from build123d import *

# Parameters (mm, degrees)
EXTRUDE_1_DEPTH     = 20
FILLET_1_R          = 2
SKETCH_2_R          = 1.5
CUT_EXTRUDE_1_DEPTH = 60.760642304
SKETCH_3_R          = 1.5
CUT_EXTRUDE_2_DEPTH = 60.760642304


with BuildPart() as part:
    # 草图1 → 凸台-拉伸1 (new body)
    with BuildSketch(Plane(origin=(0, 0, 0), x_dir=(1, 0, 0), z_dir=(0, 1, 0))):
        Polygon((0, 45), (0, 0), (40.249223595, 0), align=None)
    extrude(amount=EXTRUDE_1_DEPTH)

    # 圆角1
    fillet_1_edges = [part.edges().sort_by_distance(p)[0] for p in [
        (40.249223595, 10, 0),
        (0, 10, 0),
        (0, 10, -45),
    ]]
    fillet(fillet_1_edges, radius=FILLET_1_R)

    # 草图2 → 切除-拉伸1 (cut, through all)
    with BuildSketch(Plane.ZY):
        with Locations((-20, 15)):
            Circle(SKETCH_2_R)
        with Locations((-20, 5)):
            Circle(SKETCH_2_R)
    extrude(amount=-CUT_EXTRUDE_1_DEPTH, mode=Mode.SUBTRACT)

    # 草图3 → 切除-拉伸2 (cut, through all)
    with BuildSketch(Plane.XY):
        with Locations((15, 15)):
            Circle(SKETCH_3_R)
        with Locations((15, 5)):
            Circle(SKETCH_3_R)
    extrude(amount=-CUT_EXTRUDE_2_DEPTH, mode=Mode.SUBTRACT)


solid = part.part
Verification items for the finished model (mm, model axes). Round coordinates to 2 decimals unless told otherwise and drop trailing zeros. Write each loop counter-clockwise with the first axis right and the second up, starting at its lowest first coordinate (ties: lowest second). Pieces come first, ordered by that corner, then holes.
(1) Section check D-D (y = 15). Enter the section's corners in (x, z), plus the area to 3 significant figures.
Returned:
outline: (0, -39.76) arc R2 ccw to (3.49, -41.1) - (13.5, -29.91) - (13.5, -21.5) - (0, -21.5) - close; (0, -18.5) - (13.5, -18.5) - (13.5, 0) - (2, 0) arc R2 ccw to (0, -2) - close; (16.5, -26.55) - (21.02, -21.5) - (16.5, -21.5) - close; (16.5, -18.5) - (23.7, -18.5) - (37.27, -3.33) arc R2 ccw to (35.78, 0) - (16.5, 0) - close
area: 752 mm2
(2) Mould release check, pull along X, two halves, no side actions. Record for faces 1 (the cylindrical face through (13.5, 15.07, -24.96)), 2 (the cylindrical face through (0.57, 10.14, -0.6)), 3 (the cylindrical face through (19.29, 14.425, -18.614)), 4 (the cylindrical face through (13.5, 5.07, -24.96)): pulls with the +X half, pulls with the -X half, needs draft (parallel to the pull), parting line crosses it, or undercut.
Returned:
face 1: undercut
face 2: pulls with the -X half
face 3: needs draft
face 4: undercut
(3) Section check A-A (y = 6). Enter the section's corners in (x, z).
Returned:
outline: (0, -39.76) arc R2 ccw to (3.49, -41.1) - (13.88, -29.48) - (13.88, -21.12) - (0, -21.12) - close; (0, -18.88) - (13.88, -18.88) - (13.88, 0) - (2, 0) arc R2 ccw to (0, -2) - close; (16.12, -26.98) - (21.36, -21.12) - (16.12, -21.12) - close; (16.12, -18.88) - (23.36, -18.88) - (37.27, -3.33) arc R2 ccw to (35.78, 0) - (16.12, 0) - close
(4) Section check C-C (x = 22). Enter the section's corners in (y, z).
Returned:
outline: (0, -20.4) - (3.56, -20.4) arc R1.5 cw (long way) to (6.44, -20.4) - (13.56, -20.4) arc R1.5 cw (long way) to (16.44, -20.4) - (20, -20.4) - (20, 0) - (0, 0) - close
(5) Depth check by flat-ended pin: pin 1 Ø2.5 at (y, z) = (15, -20) entering from +X; pin 2 Ø6 at (y, z) = (12, -14) entering from +X; pin 3 Ø3 at (x, y) = (33, 15) entering from -Z; pin 4 Ø3 at (x, y) = (15.5, 12.5) entering from -Z. Enter the tip coordinate at first touch or a pass-through.
Returned:
pin 1: passes through
pin 2: stops at x = 30.41
pin 3: stops at z = -9.78
pin 4: stops at z = -29.35
(6) Section check B-B (z = -23.5). Enter the section's corners in (x, y).
Returned:
outline: (0, 0) - (19.23, 0) - (19.23, 20) - (0, 20) - close; hole circle Ø3 at (15, 5); hole circle Ø3 at (15, 15)
(7) Material ranges on line 1 (Y direction, x = 15, z = -7); line 2 (X direction, y = 12.25, z = -18.5); line 3 (X direction, y = 5.75, z = -25.5), recorded low to high.
Returned:
line 1: y = 0 to 3.5, 6.5 to 13.5, 16.5 to 20
line 2: x = 0 to 23.7
line 3: x = 0 to 13.7, 16.3 to 17.44
